Could you check a few things on this model? Use its own coordinates, in mm. Face numbers are marked on the shaded views. A direction names the side the tool comes from. Coordinates: 2 decimals unless noted, no trailing zeros. Order: outer loops, then holes, each group sorted by start corner. A loop starts at its lowest first (then second) coordinate and runs counter-clockwise, first axis right, second up. Notation, with made-up numbers: (34.5, 84.25) -> (57.5, 84.25) arc R12 cw to (57.5, 105.25) -> close; hole circle Ø4 at (81.5, -34). An arc over 180 degrees is marked (long way). Use a Markdown table: item, result. Add a question column.
1) If we section it at A-A (z = 0): Write out the boundary of the cut face in (x, y), plus the area to 3 significant figures.
2) If we section it at C-C (y = -20): Write out the boundary of the cut face in (x, z).
3) Will these pins go through, and if not, where does the flat tip stop? pin 1 Ø3 at (x, y) = (-1, -15.5) entering from -Z; pin 2 Ø6 at (x, y) = (-1, 21.5) entering from +Z; pin 3 Ø4 at (y, z) = (-23, 3.5) entering from -X.
4) Which directions (+Z, -Z, +X, -X, +Y, -Y) give clear straight access to the entire face, cutting with the end or side of a thin tool? Please do the marked faces 1 and 2.
5) If I drill on L1, parallel to Y at x = 1, z = 0; L2, parallel to Y at x = -3.25, z = -15.5; L3, parallel to Z at x = -0.5, y = 2, over which ranges is the centre line in solid material (lowest first)? Write a range as [from, to].
6) Thinking about a two-plate mould opening in Z: for the marked faces 3, 4 and 5, which applies, +Z half, -Z half, draft (parallel to the pull), parting line (faces both ways), or undercut?
7) If we section it at D-D (x = -3): Write out the boundary of the cut face in (y, z).
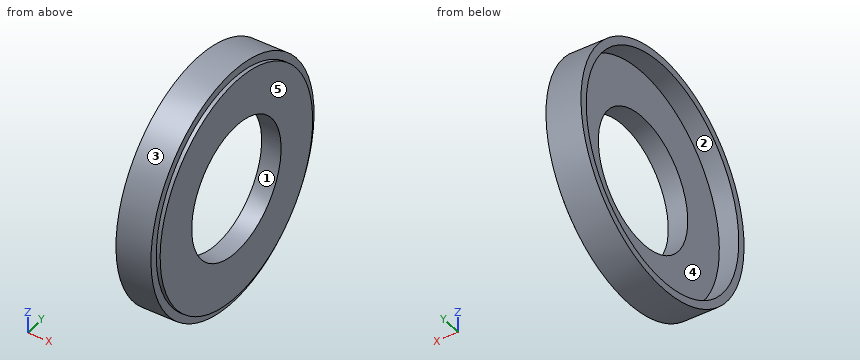
```python
from build123d import *


with BuildPart() as part:
    # 草图1 → 旋转1 (revolve)
    with BuildSketch(Plane.XY, mode=Mode.PRIVATE) as revolve_1_sk:
        Polygon((-1.646669205, 17), (3.353330795, 17), (3.353330795, 29), (2.353330795, 29), (2.353330795, 31), (-6.646669205, 31), (-6.646669205, 29), (-1.646669205, 29), align=None)
    revolve(revolve_1_sk.sketch.rotate(Axis((0, 0, 0), (1, 0, 0)), 90), axis=Axis((0, 0, 0), (1, 0, 0)))


solid = part.part
```
Answer sheet:
| question | item | result |
|---|---|---|
| 1 | outline | (-6.65, -31) -> (2.35, -31) -> (2.35, -29) -> (3.35, -29) -> (3.35, -17) -> (-1.65, -17) -> (-1.65, -29) -> (-6.65, -29) -> close; (-6.65, 29) -> (-1.65, 29) -> (-1.65, 17) -> (3.35, 17) -> (3.35, 29) -> (2.35, 29) -> (2.35, 31) -> (-6.65, 31) -> close |
| 1 | area | 156 mm2 |
| 2 | outline | (-6.65, -23.69) -> (2.35, -23.69) -> (2.35, -21) -> (3.35, -21) -> (3.35, 21) -> (2.35, 21) -> (2.35, 23.69) -> (-6.65, 23.69) -> (-6.65, 21) -> (-1.65, 21) -> (-1.65, -21) -> (-6.65, -21) -> close |
| 3 | pin 1 | z = -27.66 |
| 3 | pin 2 | z = 24.87 |
| 3 | pin 3 | x = -1.65 |
| 4 | face 1 | +X, -X |
| 4 | face 2 | -X |
| 5 | L1 | [-31, -17], [17, 31] |
| 5 | L2 | [-26.85, -24.51], [24.51, 26.85] |
| 5 | L3 | [-30.94, -16.88], [16.88, 30.94] |
| 6 | face 3 | parting line |
| 6 | face 4 | undercut |
| 6 | face 5 | draft |
| 7 | outline | circle Ø62 at (0, 0); hole circle Ø58 at (0, 0) |
